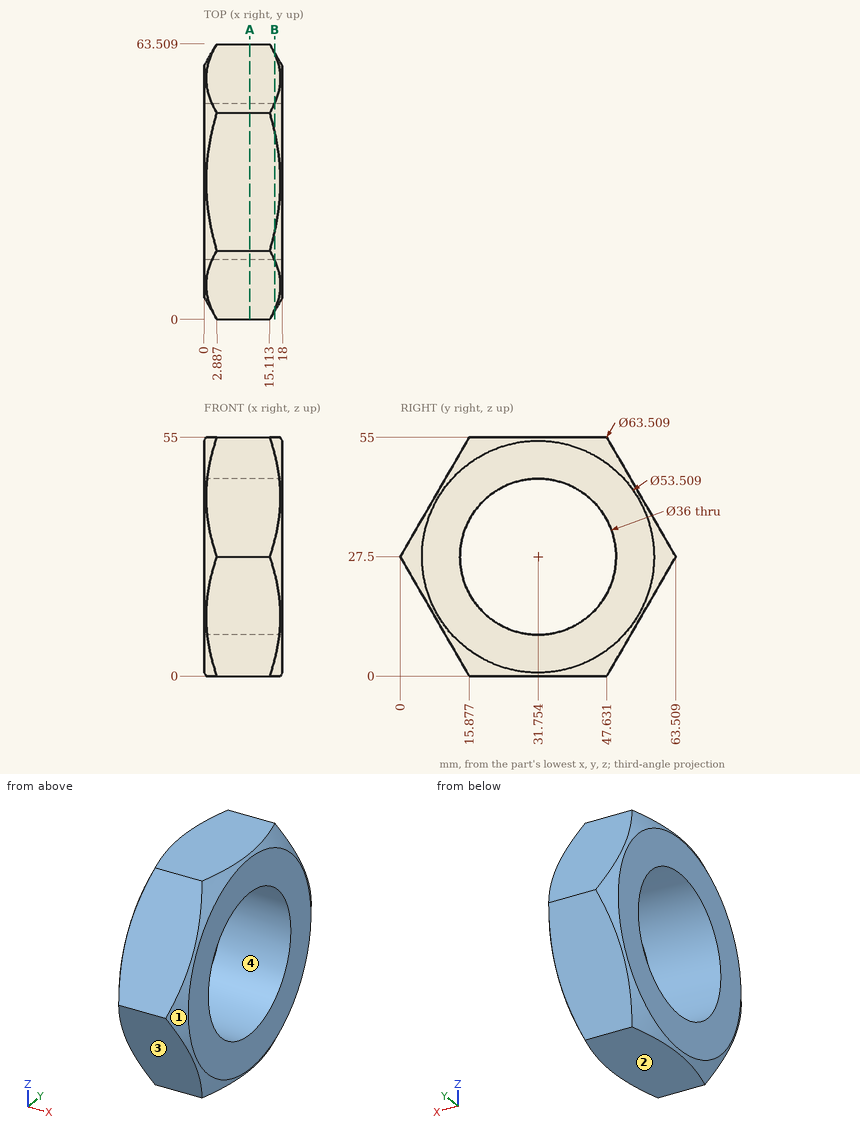
Answer from the drawing. Dimensions are ordinates in mm from the lowest x, y and z of the part. Round coordinates to 2 decimals unless told otherwise and drop trailing zeros. Loops run counter-clockwise (first coordinate to the right, second up) from the corner with the lowest first, then second, coordinate; pieces in that order, holes last.
1) A cutting plane is placed at B-B on x = 16.25. Determine the outline of the cut face in (y, z) (1 decimal).
Outcome:
outline: (2.2, 23.7) - (13.7, 3.8) arc R29.8 ccw to (20.3, 0) - (43.2, 0) arc R29.8 ccw to (49.8, 3.8) - (61.3, 23.7) arc R29.8 ccw to (61.3, 31.3) - (49.8, 51.2) arc R29.8 ccw to (43.2, 55) - (20.3, 55) arc R29.8 ccw to (13.7, 51.2) - (2.2, 31.3) arc R29.8 ccw to start; hole circle Ø36 at (31.8, 27.5)
2) Given P1, Ø2, axis at x = 10, z = 13.5, coming from the +Y side; P2, Ø10, axis at x = 15, y = 56.5, coming from the +Z side, each flat-ended and moving along its own axis, determine where each tip first touches the part or whether it passes through.
Outcome:
P1: stops at y = 56
P2: stops at z = 48.3
3) For a pull along Y with two mould halves and no side action, classify the marked faces 1, 2, 3 and 4 as released by +Y, released by -Y, zero draft, split by the parting line, or undercut.
Outcome:
face 1: split by the parting line
face 2: zero draft
face 3: released by -Y
face 4: undercut
4) Consider line 1 (Z direction, x = 10, y = 23); line 2 (Y direction, x = 2.5, z = 19); line 3 (Z direction, x = 1.75, y = 39). Determine where each line is inside the solid, lowest interval first.
Outcome:
line 1: z = 0 to 11.77, 43.23 to 55
line 2: y = 4.91 to 15.89, 47.62 to 58.6
line 3: z = 0 to 11.02, 43.98 to 55
5) A cutting plane is placed at A-A on x = 10.5. Determine the outline of the cut face in (y, z) (1 decimal), plus the area to 3 significant figures.
Outcome:
outline: (0, 27.5) - (15.9, 0) - (47.6, 0) - (63.5, 27.5) - (47.6, 55) - (15.9, 55) - close; hole circle Ø36 at (31.8, 27.5)
area: 1,600 mm2
